```python
from build123d import *

# Parameters (mm, degrees)
CHAMFER1_SIZE           = 0.2
CUT_EXTRUDE2_DEPTH      = 30.69848481
CUT_EXTRUDE2_DEPTH_BACK = 30.69848481
SKETCH3_R               = 1.5
CHAMFER2_SIZE           = 0.2


with BuildPart() as part:
    # Sketch1 → Revolve1 (revolve)
    with BuildSketch(Plane.XY, mode=Mode.PRIVATE) as revolve1_sk:
        Polygon((0, 0), (0, 5), (10, 5), (10, 7), (28, 7), (28, 0), align=None)
    revolve(revolve1_sk.sketch.rotate(Axis((0, 0, 0), (1, 0, 0)), 90), axis=Axis((0, 0, 0), (1, 0, 0)))

    # Chamfer1
    chamfer1_edges = [part.edges().sort_by_distance(p)[0] for p in [
        (0, 0, -5),
    ]]
    chamfer(chamfer1_edges, length=CHAMFER1_SIZE)

    # Sketch3 → Cut-Extrude2 (cut, two sides: drawn at the far end of the back side and taken through both)
    with BuildSketch(Plane(origin=(0, 0, 0), x_dir=(1, 0, 0), z_dir=(0, 1, 0)).offset(-CUT_EXTRUDE2_DEPTH_BACK)):
        with Locations(Location((25, 0, 0), (0, 0, 270))):
            Circle(SKETCH3_R)
    extrude(amount=CUT_EXTRUDE2_DEPTH + CUT_EXTRUDE2_DEPTH_BACK, mode=Mode.SUBTRACT)

    # Chamfer2
    chamfer2_edges = [part.edges().sort_by_distance(p)[0] for p in [
        (28, 0, -7),
    ]]
    chamfer(chamfer2_edges, length=CHAMFER2_SIZE)


solid = part.part
```
Read the model definition and answer for the solid it produces. Units are mm, in the model's axes. A direction names the side the tool comes from. Coordinates: 2 decimals unless noted, no trailing zeros. Write each loop counter-clockwise with the first axis right and the second up, starting at its lowest first coordinate (ties: lowest second). Pieces come first, ordered by that corner, then holes. Notation, with made-up numbers: (59.5, 40) - (65.5, 40) arc R14 cw to (65.5, 65) - close; hole circle Ø5 at (41, 1). An arc over 180 degrees is marked (long way). Answer as a JSON object with one key per item and string values. Group by question number.
1. Each of these flat-tipped pins is pushed along its axis until it touches: P1, Ø8, axis at x = 8, y = 4, coming from the +Z side; P2, Ø1, axis at x = 12, z = 1.5, coming from the +Y side. Where does it stop, or does it pass through?
2. A cutting plane is placed at D-D (x = 15.5). Determine the outline of the cut face in (y, z), plus the area to 3 significant figures.
3. A cutting plane is placed at A-A (y = 0). Determine the outline of the cut face in (x, z).
4. Consider L1, parallel to X at y = 3.5, z = 0; L2, parallel to Z at x = 6.5, y = 0.25; L3, parallel to X at y = -2.5, z = 4.75. Determine where each line is inside the solid, lowest interval first. Write a range as [from, to].
5. A cutting plane is placed at B-B (z = 0). Determine the outline of the cut face in (x, y), plus the area to 3 significant figures.
6. The mould has two halves that part along X. Classify faces 1 (the flat face through (0, 0, 0)), 2 (the cylindrical face through (26.487, -0.098, -0.195)), 3 (the flat face through (28, 0, 0)): +X half, -X half, draft (parallel to the pull), parting line (faces both ways), or undercut.
7. Which of the six approach directions +Z, -Z, +X, -X, +Y, -Y give full straight-line access (tool end or side, diameter ignored) to faces 4 (the cylindrical face through (5, 0, -5)), 5 (the cylindrical face through (19.025, 6.834, -1.517))?
8. A cutting plane is placed at C-C (x = 7). Determine the outline of the cut face in (y, z).
Worked out:
{
 "1": {"P1": "stops at z = 6.98", "P2": "stops at y = 6.93"},
 "2": {"outline": "circle Ø14 at (0, 0)", "area": "154 mm²"},
 "3": {"outline": "(0, -4.8) - (0.2, -5) - (10, -5) - (10, -7) - (27.8, -7) - (28, -6.8) - (28, 6.8) - (27.8, 7) - (10, 7) - (10, 5) - (0.2, 5) - (0, 4.8) - close; hole circle Ø3 at (25, 0)"},
 "4": {"L1": "x = [0, 23.5], [26.5, 28]", "L2": "z = [-4.99, 4.99]", "L3": "x = [10, 28]"},
 "5": {"outline": "(0, -4.8) - (0.2, -5) - (10, -5) - (10, -7) - (23.5, -7) - (23.5, 7) - (10, 7) - (10, 5) - (0.2, 5) - (0, 4.8) - close; (26.5, -7) - (27.8, -7) - (28, -6.8) - (28, 6.8) - (27.8, 7) - (26.5, 7) - close", "area": "310 mm²"},
 "6": {"face 1": "-X half", "face 2": "undercut", "face 3": "+X half"},
 "7": {"face 4": "-X", "face 5": "+X, -X"},
 "8": {"outline": "circle Ø10 at (0, 0)"}
}
